Input: part model. Units: mm. Frame: model coordinates. Face numbers are marked on the shaded views. Round coordinates to 2 decimals unless told otherwise and drop trailing zeros. Write each loop counter-clockwise with the first axis right and the second up, starting at its lowest first coordinate (ties: lowest second). Pieces come first, ordered by that corner, then holes. Notation, with made-up numbers: M 88,13.25 L 143,13.25 A13 ccw 143,20.25 Z; hole C 71.25,36 d8. An arc over 180 degrees is marked long. Write each question's results on one line, items separated by ' | '. Start each with the question number.
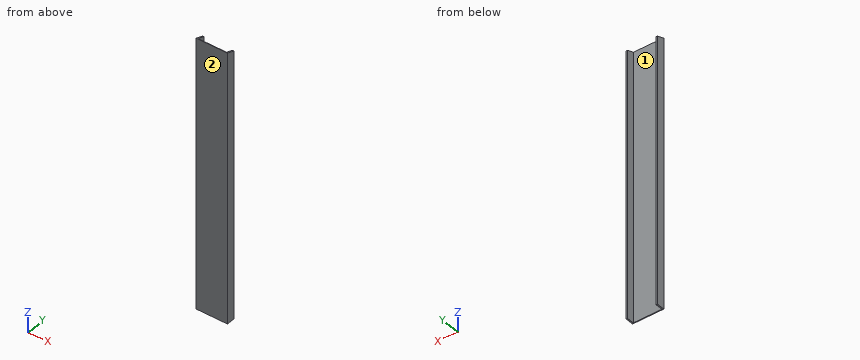
```python
from build123d import *

# Parameters (mm, degrees)
BOSS_EXTRUDE1_DEPTH = 1099.3375
CUT_EXTRUDE1_DEPTH  = 150


with BuildPart() as part:
    # Sketch1 → Boss-Extrude1 (new, symmetric)
    with BuildSketch(Plane.XY):
        Polygon((127, 0), (-127, 0), (-127, 66.04), (-115.9256, 66.04), (-115.9256, 6.096), (115.9256, 6.096), (115.9256, 66.04), (127, 66.04), align=None)
    extrude(amount=BOSS_EXTRUDE1_DEPTH, both=True)

    # Sketch2 → Cut-Extrude1 (cut, symmetric)
    with BuildSketch(Plane(origin=(0, 0, 0), x_dir=(0, 0, -1), z_dir=(1, 0, 0))):
        Polygon((-1099.3375, 0), (-1076.752705704, 66.04), (-1099.3375, 66.04), align=None)
    extrude(amount=CUT_EXTRUDE1_DEPTH, both=True, mode=Mode.SUBTRACT)


solid = part.part
```
1. Cut plane B-B on y = 41. Output: boundary loops of the cut face in (x, z), and give its area (3 significant figures).
2. Contact query for a flat-ended pin moving along its axis: P1, Ø5, axis at x = -64, z = 455.5, coming from the +Y side. Output: stop coordinate, or through.
3. Cut plane C-C on x = -49. Output: boundary loops of the cut face in (y, z).
4. Draft query along X for the marked faces 1 and 2. Return one class per face: +X half, -X half, draft (parallel to the pull), parting line (faces both ways), or undercut.
5. Cut plane A-A on z = -98.5. Output: boundary loops of the cut face in (x, y).
6. Line query: L1, parallel to X at y = 59, z = -596.5; L2, parallel to Y at x = -105.5, z = -92.5. Output: solid intervals per line, ascending. Write a range as from..to.
Answers follow:
1) outline: M -127,-1099.34 L -115.93,-1099.34 L -115.93,1085.32 L -127,1085.32 Z; M 115.93,-1099.34 L 127,-1099.34 L 127,1085.32 L 115.93,1085.32 Z | area: 48,400 mm2
2) P1: stops at y = 6.1
3) outline: M 0,-1099.34 L 6.1,-1099.34 L 6.1,1097.25 L 0,1099.34 Z
4) face 1: undercut | face 2: draft
5) outline: M -127,0 L 127,0 L 127,66.04 L 115.93,66.04 L 115.93,6.1 L -115.93,6.1 L -115.93,66.04 L -127,66.04 Z
6) L1: x = -127..-115.93, 115.93..127 | L2: y = 0..6.1
